Input: dimensioned drawing with shaded views. Units: mm. Origin: part minimum x, y, z. A direction names the side the tool comes from. Give positions to 0.01 mm unless a question says otherwise; leave off trailing zeros. Loops run counter-clockwise (first coordinate to the right, second up) from the corner with the lowest first, then second, coordinate; pieces in that order, holes last.
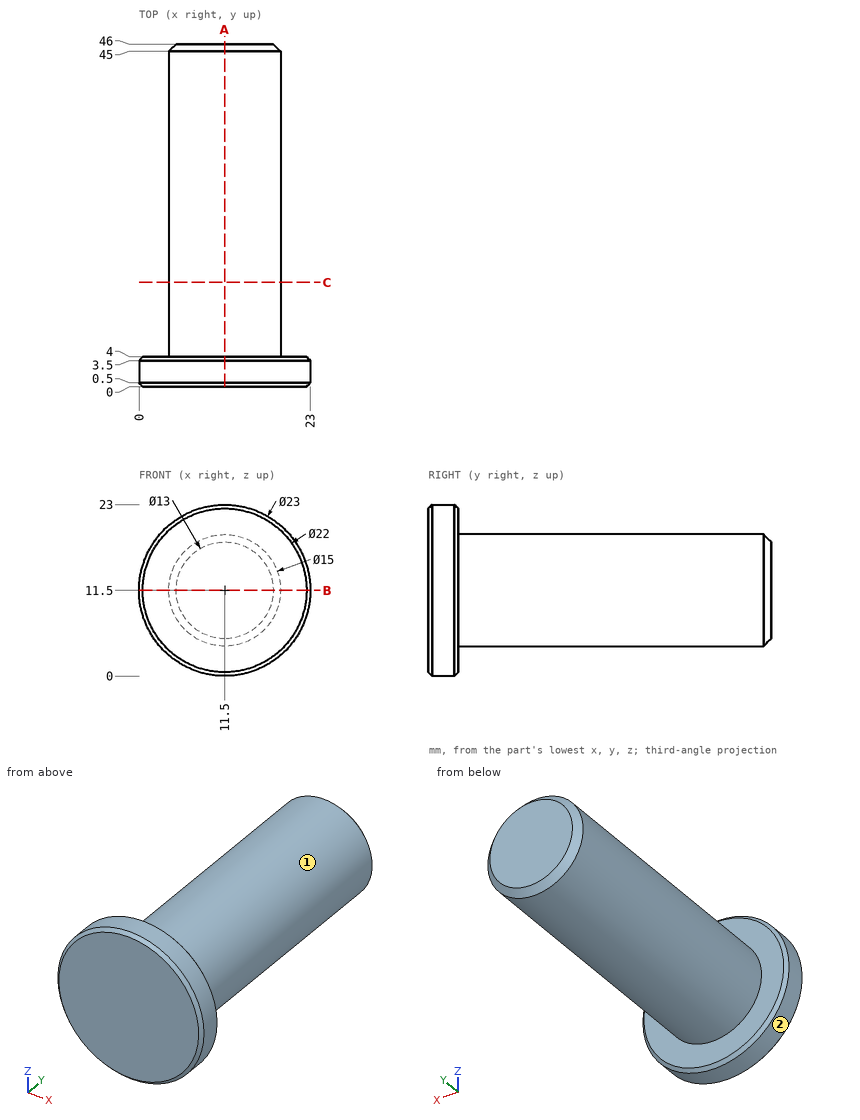
(1) Ray query, line 1 along Y through (x, z) = (7, 2.75); line 2 along Z through (x, y) = (15.25, 15); line 3 along Z through (x, y) = (12.5, 43). Return the intervals inside material, ascending.
A:
line 1: y = 0 to 4
line 2: z = 5 to 18
line 3: z = 4.07 to 18.93
(2) Section C-C, the plane y = 14. Return the cut outline in (x, z), then the cut area to 3 significant figures.
A:
outline: circle Ø15 at (11.5, 11.5)
area: 177 mm2
(3) Section A-A, the plane x = 11.5. Return the cut outline in (y, z), then the cut area to 4 significant figures.
A:
outline: (0, 0.5) - (0.5, 0) - (3.5, 0) - (4, 0.5) - (4, 4) - (45, 4) - (46, 5) - (46, 18) - (45, 19) - (4, 19) - (4, 22.5) - (3.5, 23) - (0.5, 23) - (0, 22.5) - close
area: 720.5 mm2
(4) First-contact query: pin 1 (8 mm diameter, centred on x = 17, y = 11, fed in from +Z); pin 2 (4 mm diameter, centred on x = 9, z = 7, fed in from -Y); pin 3 (12 mm diameter, centred on x = 3, y = 22.5, fed in from +Z); pin 4 (3 mm diameter, centred on y = 11, z = 15, fed in from +X). Flat tips, straight axial feed; report the tip coordinate or a pass-through.
A:
pin 1: stops at z = 18.85
pin 2: stops at y = 0
pin 3: stops at z = 18.57
pin 4: stops at x = 18.73
(5) Reachability of the marked faces 1 and 2 from +Z, -Z, +X, -X, +Y, -Y: full face, straight path, thin tool, end or side. Return the list, or none.
A:
face 1: +Y
face 2: +Y, -Y
(6) Section B-B, the plane z = 11.5. Return the cut outline in (x, y), then the cut area to 4 significant figures.
A:
outline: (0, 0.5) - (0.5, 0) - (22.5, 0) - (23, 0.5) - (23, 3.5) - (22.5, 4) - (19, 4) - (19, 45) - (18, 46) - (5, 46) - (4, 45) - (4, 4) - (0.5, 4) - (0, 3.5) - close
area: 720.5 mm2
